Here's how the part is built. I have some questions about the finished solid (model axes, mm). Face numbers are marked on the shaded views. A direction names the side the tool comes from. Coordinates: 2 decimals unless noted, no trailing zeros. Order: outer loops, then holes, each group sorted by start corner. A loop starts at its lowest first (then second) coordinate and runs counter-clockwise, first axis right, second up. Notation, with made-up numbers: (71, -15) - (126, -15) arc R7 ccw to (126, -6) - close; hole circle Ø4 at (-7.75, 53). An arc over 180 degrees is marked (long way). Answer in a Markdown table with one row per item. Add a question column.
Item 1: I want a section at D-D (z = -92.5). Please give me the cut outline in (x, y), plus the area to 3 significant figures.
Item 2: If I drill on line 1 along X through (y, z) = (51.5, -89); line 2 along Z through (x, y) = (-9.5, 18); line 3 along Y through (x, z) = (-15.5, -64), over which ranges is the centre line in solid material (lowest first)? Write a range as from..to.
Item 3: Will these pins go through, and if not, where does the flat tip stop? pin 1 Ø12 at (x, z) = (-13, -76.5) entering from -Y; pin 2 Ø15 at (x, y) = (2, 8) entering from -Z.
Item 4: On a 3-axis mill with a long thin cutter (end or side, diameter ignored), from which of +Z, -Z, +X, -X, +Y, -Y can I reach the whole of each face in a straight line? I mean the marked faces 1 and 2. Say none if no direction works.
Item 5: I want a section at A-A (y = 26). Please give me the cut outline in (x, z), plus the area to 3 significant figures.
Item 6: I want a section at C-C (x = 21.5). Please give me the cut outline in (y, z), plus the area to 4 significant figures.
Item 7: I want a section at B-B (z = -15.5). Please give me the cut outline in (x, y), plus the area to 3 significant figures.
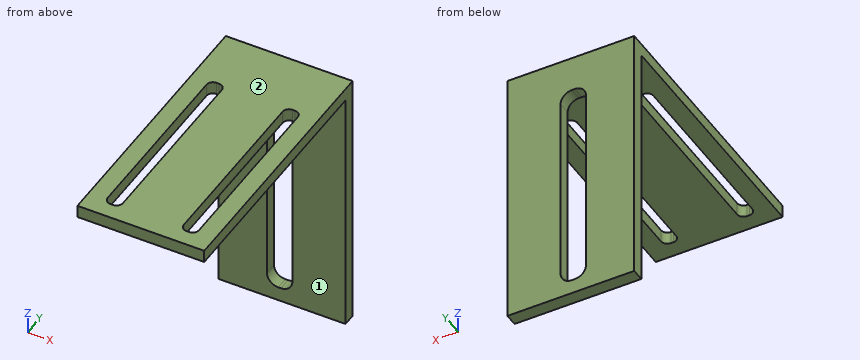
```python
from build123d import *

# Parameters (mm, degrees)
SKETCH1_W                = 50
SKETCH1_H                = 100
BOSS_EXTRUDE1_DEPTH      = 5
CUT_EXTRUDE1_DEPTH       = 10
BOSS_EXTRUDE2_DEPTH      = 100
BOSS_EXTRUDE2_DEPTH_BACK = 5
SKETCH4_W                = 50
SKETCH4_H                = 5
CUT_EXTRUDE3_DEPTH       = 80


with BuildPart() as part:
    # Sketch1 → Boss-Extrude1 (new body)
    with BuildSketch(Plane.XY):
        Rectangle(SKETCH1_W, SKETCH1_H)
    extrude(amount=BOSS_EXTRUDE1_DEPTH)

    # Sketch2 → Cut-Extrude1 (cut)
    with BuildSketch(Plane.XY.offset(5)):
        with BuildLine():
            Line((-14.5, -43.655057898), (-15.5, -43.655057898))
            ThreePointArc((-15.5, -43.655057898), (-17.267766953, -42.922824851), (-18, -41.155057898))
            Line((-18, -41.155057898), (-18, 28.844942102))
            ThreePointArc((-18, 28.844942102), (-17.267766953, 30.612709055), (-15.5, 31.344942102))
            Line((-15.5, 31.344942102), (-14.5, 31.344942102))
            ThreePointArc((-14.5, 31.344942102), (-12.732233047, 30.612709055), (-12, 28.844942102))
            Line((-12, 28.844942102), (-12, -41.155057898))
            ThreePointArc((-12, -41.155057898), (-12.732233047, -42.922824851), (-14.5, -43.655057898))
        make_face()
        with BuildLine():
            Line((15.5, -43.655057898), (14.5, -43.655057898))
            ThreePointArc((14.5, -43.655057898), (12.732233047, -42.922824851), (12, -41.155057898))
            Line((12, -41.155057898), (12, 28.844942102))
            ThreePointArc((12, 28.844942102), (12.732233047, 30.612709055), (14.5, 31.344942102))
            Line((14.5, 31.344942102), (15.5, 31.344942102))
            ThreePointArc((15.5, 31.344942102), (17.267766953, 30.612709055), (18, 28.844942102))
            Line((18, 28.844942102), (18, -41.155057898))
            ThreePointArc((18, -41.155057898), (17.267766953, -42.922824851), (15.5, -43.655057898))
        make_face()
    extrude(amount=-CUT_EXTRUDE1_DEPTH, mode=Mode.SUBTRACT)

    # Sketch4 → Boss-Extrude2 (add, two sides: drawn at the far end of the back side and taken through both)
    with BuildSketch(Plane(origin=(0, 0, 0), x_dir=(-1, 0, 0), z_dir=(0, 0, -1)).offset(-BOSS_EXTRUDE2_DEPTH_BACK)):
        with Locations((0, 52.5)):
            Rectangle(SKETCH4_W, SKETCH4_H)
    extrude(amount=BOSS_EXTRUDE2_DEPTH + BOSS_EXTRUDE2_DEPTH_BACK)

    # Sketch5 → Cut-Extrude3 (cut)
    with BuildSketch(Plane.XZ.offset(-50)):
        with BuildLine():
            Line((-0.473985761, -94.252877225), (-1.473985761, -94.252877225))
            ThreePointArc((-1.473985761, -94.252877225), (-4.655966276, -92.934857741), (-5.973985761, -89.752877225))
            Line((-5.973985761, -89.752877225), (-5.973985761, -13.752877225))
            ThreePointArc((-5.973985761, -13.752877225), (-4.655966276, -10.57089671), (-1.473985761, -9.252877225))
            Line((-1.473985761, -9.252877225), (-0.473985761, -9.252877225))
            ThreePointArc((-0.473985761, -9.252877225), (2.707994755, -10.57089671), (4.026014239, -13.752877225))
            Line((4.026014239, -13.752877225), (4.026014239, -89.752877225))
            ThreePointArc((4.026014239, -89.752877225), (2.707994755, -92.934857741), (-0.473985761, -94.252877225))
        make_face()
    extrude(amount=-CUT_EXTRUDE3_DEPTH, mode=Mode.SUBTRACT)


solid = part.part
```
Values follow:
| question | item | result |
|---|---|---|
| 1 | outline | (-25, 50) - (-5.04, 50) - (-5.04, 55) - (-25, 55) - close; (3.09, 50) - (25, 50) - (25, 55) - (3.09, 55) - close |
| 1 | area | 209 mm^2 |
| 2 | line 1 | x = -25..-5.97, 4.03..25 |
| 2 | line 2 | z = 0..5 |
| 2 | line 3 | y = 50..55 |
| 3 | pin 1 | stops at y = 50 |
| 3 | pin 2 | stops at z = 0 |
| 4 | face 1 | -Z, +X, -X, -Y |
| 4 | face 2 | +Z, +X, -X, +Y, -Y |
| 5 | outline | (-25, 0) - (-18, 0) - (-18, 5) - (-25, 5) - close; (-12, 0) - (12, 0) - (12, 5) - (-12, 5) - close; (18, 0) - (25, 0) - (25, 5) - (18, 5) - close |
| 5 | area | 190 mm^2 |
| 6 | outline | (-50, 0) - (50, 0) - (50, -100) - (55, -100) - (55, 5) - (-50, 5) - close |
| 6 | area | 1,025 mm^2 |
| 7 | outline | (-25, 50) - (-5.97, 50) - (-5.97, 55) - (-25, 55) - close; (4.03, 50) - (25, 50) - (25, 55) - (4.03, 55) - close |
| 7 | area | 200 mm^2 |
